Study the drawing (mm; zero at the part's minimum x, y, z) and answer. A direction names the side the tool comes from. Give positions to 0.01 mm unless a question says otherwise; leave off trailing zeros. Order: outer loops, then holes, each group sorted by start corner. A loop starts at its lowest first (then second) coordinate and runs counter-clockwise, first axis right, second up.
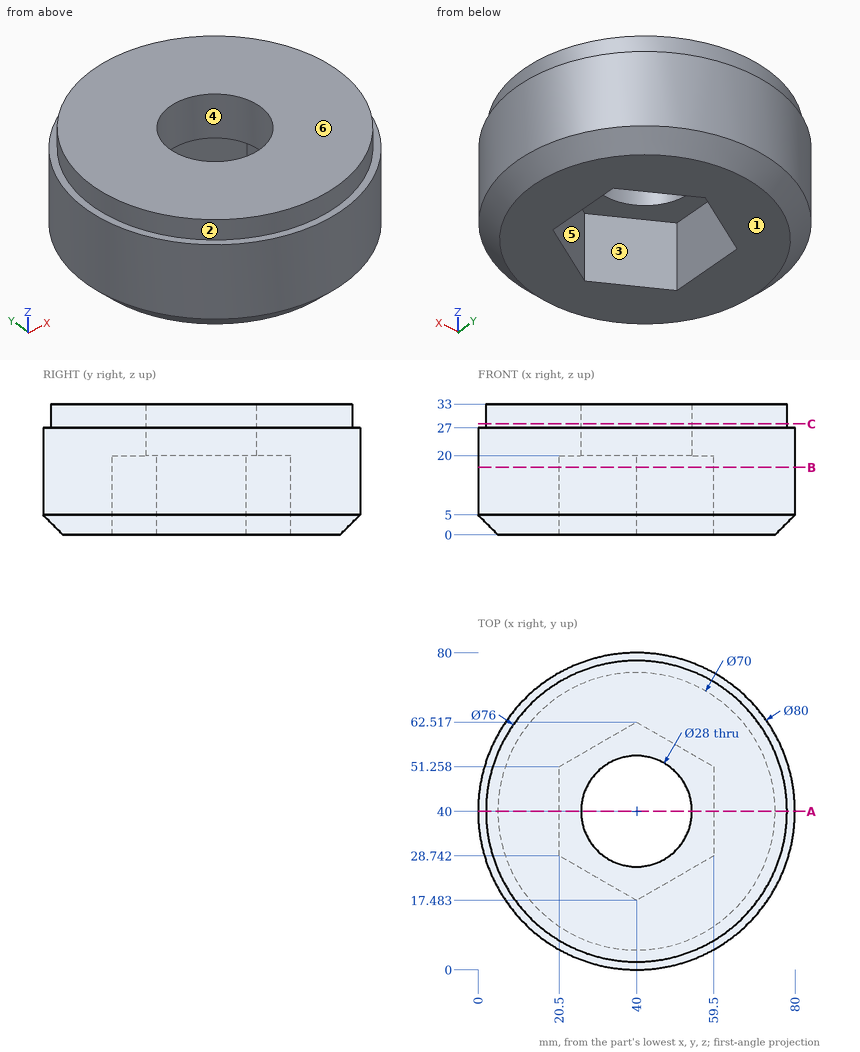
1) Find section B-B (z = 17). Write down the section's boundary in (x, y), then the cut area to 3 significant figures.
Geometry says:
outline: circle Ø80 at (40, 40); hole (20.5, 28.74) - (40, 17.48) - (59.5, 28.74) - (59.5, 51.26) - (40, 62.52) - (20.5, 51.26) - close
area: 3,710 mm2
2) Given P1, Ø11.5, axis at x = 33, y = 48, coming from the -Z side; P2, Ø1, axis at y = 39, z = 23.5, coming from the +X side; P3, Ø3, axis at y = 58.5, z = 13.5, coming from the -X side, each flat-ended and moving along its own axis, determine where each tip first touches the part or whether it passes through.
Geometry says:
P1: stops at z = 20
P2: stops at x = 80
P3: stops at x = 3.79
3) For a pull along Y with two mould halves and no side action, classify the marked faces 1, 2, 3 and 4 as +Y half, -Y half, draft (parallel to the pull), parting line (faces both ways), or undercut.
Geometry says:
face 1: draft
face 2: parting line
face 3: undercut
face 4: undercut
4) Find section A-A (y = 40). Write down the section's boundary in (x, z), then the cut area to 3 significant figures.
Geometry says:
outline: (0, 5) - (5, 0) - (20.5, 0) - (20.5, 20) - (26, 20) - (26, 33) - (2, 33) - (2, 27) - (0, 27) - close; (54, 20) - (59.5, 20) - (59.5, 0) - (75, 0) - (80, 5) - (80, 27) - (78, 27) - (78, 33) - (54, 33) - close
area: 1,450 mm2
5) A tool of negligible diameter and unlimited length cuts with its end or side. For the marked faces 5 and 6, from which of +Z, -Z, +X, -X, +Y, -Y can it reach the whole face along a straight path? Write none if from no direction.
Geometry says:
face 5: -Z
face 6: +Z, +X, -X, +Y, -Y
6) Straight lines are drawn through the part: probe 1 along Y at (x, z) = (40, 26.25); probe 2 along Y at (x, z) = (40, 29); probe 3 along X at (y, z) = (53, 31) (1 decimal). For each, find the intervals that lie inside material, in ascending order.
Geometry says:
probe 1: y = 0 to 26, 54 to 80
probe 2: y = 2 to 26, 54 to 78
probe 3: x = 4.3 to 34.8, 45.2 to 75.7
7) Find section C-C (z = 28). Write down the section's boundary in (x, y), then the cut area to 3 significant figures.
Geometry says:
outline: circle Ø76 at (40, 40); hole circle Ø28 at (40, 40)
area: 3,920 mm2
